Input: dimensioned drawing with shaded views. Units: mm. Origin: part minimum x, y, z. Round coordinates to 2 decimals unless told otherwise and drop trailing zeros. Loops run counter-clockwise (first coordinate to the right, second up) from the corner with the lowest first, then second, coordinate; pieces in that order, holes last. Notation, with made-up numbers: M -13,48.25 L 31,48.25 A22 cw 31,75.25 Z; hole C -22.75,25.5 d7. An arc over 180 degrees is marked long. Write each question's results on one line, items separated by ' | '. Start each with the question number.
1. Draft query along Y for the marked faces 1, 2, 3 and 4. Return one class per face: released by +Y, released by -Y, zero draft, split by the parting line, or undercut.
2. Section B-B on z = 2. Output: boundary loops of the cut face in (x, y), and give its area (3 significant figures).
3. Section D-D on x = 4.5. Output: boundary loops of the cut face in (y, z).
4. Ray query, line 1 (Y direction, x = 15, z = 2.5); line 2 (Y direction, x = 13, z = 3); line 3 (Y direction, x = 28.75, z = 7) (1 decimal). Return the intervals inside material, ascending.
5. Section A-A on x = 15. Output: boundary loops of the cut face in (y, z), and give its area (3 significant figures).
6. Section C-C on x = 26.5. Output: boundary loops of the cut face in (y, z) (1 decimal).
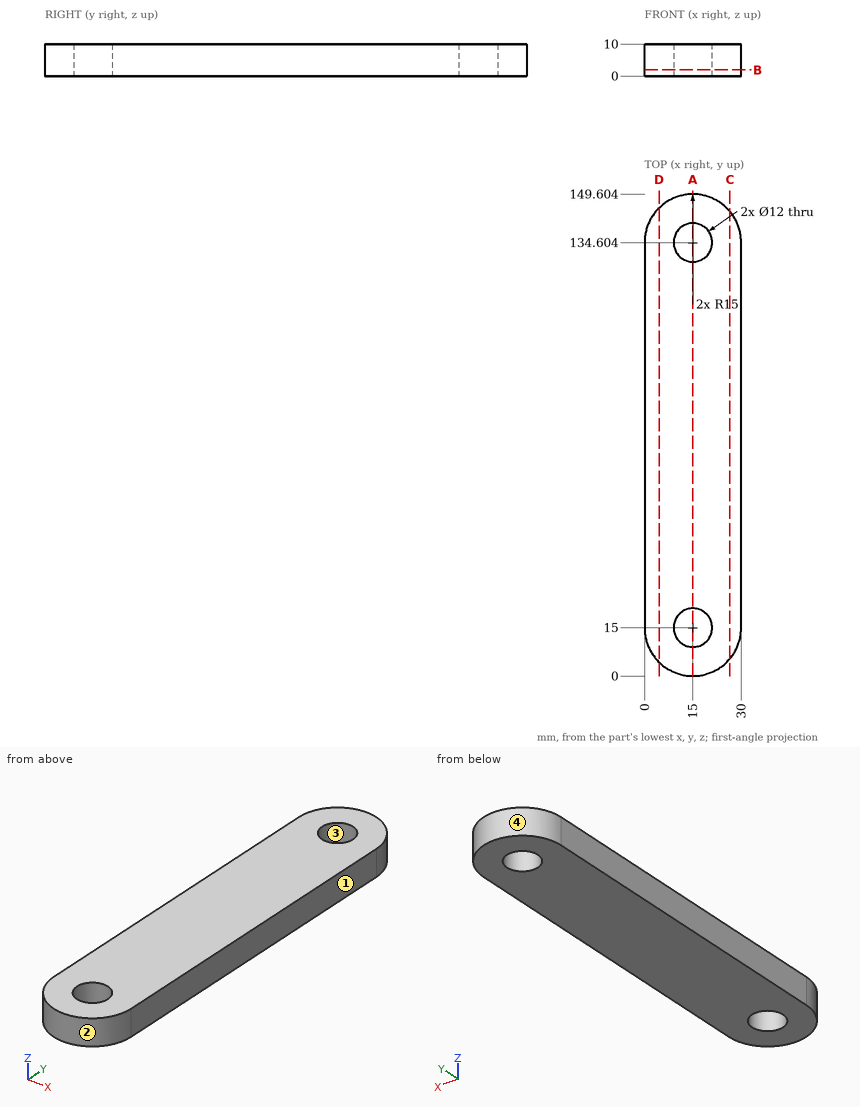
Taken from the geometry:
1) face 1: zero draft | face 2: released by -Y | face 3: undercut | face 4: released by +Y
2) outline: M 0,15 A15 ccw 30,15 L 30,134.6 A15 ccw 0,134.6 Z; hole C 15,15 d12; hole C 15,134.6 d12 | area: 4,070 mm^2
3) outline: M 4.29,0 L 145.32,0 L 145.32,10 L 4.29,10 Z
4) line 1: 0 to 9, 21 to 128.6, 140.6 to 149.6 | line 2: 0.13 to 9.34, 20.66 to 128.95, 140.26 to 149.47 | line 3: 9 to 140.6
5) outline: M 0,0 L 9,0 L 9,10 L 0,10 Z; M 21,0 L 128.6,0 L 128.6,10 L 21,10 Z; M 140.6,0 L 149.6,0 L 149.6,10 L 140.6,10 Z | area: 1,260 mm^2
6) outline: M 5.4,0 L 144.2,0 L 144.2,10 L 5.4,10 Z
